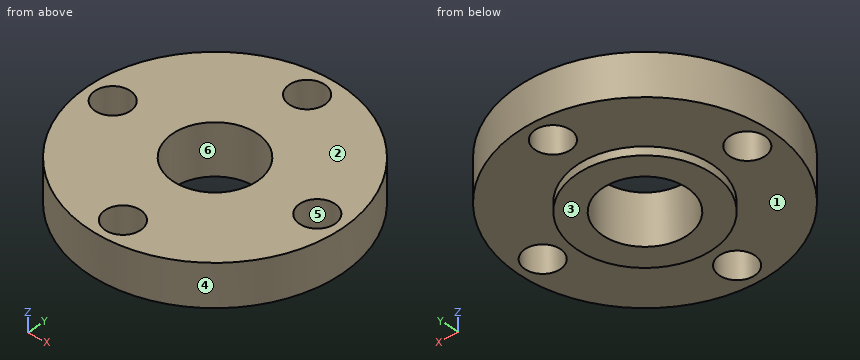
```python
from build123d import *

# Parameters (mm, degrees)
SKETCH1_R           = 15
BOSS_EXTRUDE1_DEPTH = 5
SKETCH2_R           = 2.1
CUT_EXTRUDE1_DEPTH  = 22.794494718
CIRPATTERN1_COUNT   = 4
SKETCH3_R           = 8
BOSS_EXTRUDE2_DEPTH = 1
SKETCH4_R           = 5
CUT_EXTRUDE3_DEPTH  = 23.045407685


with BuildPart() as part:
    # Sketch1 → Boss-Extrude1 (new body)
    with BuildSketch(Plane.XY):
        Circle(SKETCH1_R)
    extrude(amount=BOSS_EXTRUDE1_DEPTH)

    # Sketch2 → Cut-Extrude1 (cut, through all)
    with BuildSketch(Plane.XY.offset(5)):
        with Locations((0, 12)):
            Circle(SKETCH2_R)
    cut_extrude1 = extrude(amount=-CUT_EXTRUDE1_DEPTH, mode=Mode.SUBTRACT)

    # CirPattern1: Cut-Extrude1 ×4 about axis
    cirpattern1_axis = Axis((0, 0, 0), (0, 0, 1))
    for i in range(1, CIRPATTERN1_COUNT):
        add(cut_extrude1.rotate(cirpattern1_axis, i * 360 / CIRPATTERN1_COUNT), mode=Mode.SUBTRACT)

    # Sketch3 → Boss-Extrude2 (add)
    with BuildSketch(Plane(origin=(0, 0, 0), x_dir=(-1, 0, 0), z_dir=(0, 0, -1))):
        with Locations(Location((0, 0, 0), (0, 0, 180))):
            Circle(SKETCH3_R)
    extrude(amount=BOSS_EXTRUDE2_DEPTH)

    # Sketch4 → Cut-Extrude3 (cut, through all)
    with BuildSketch(Plane.XY.offset(5)):
        Circle(SKETCH4_R)
    extrude(amount=-CUT_EXTRUDE3_DEPTH, mode=Mode.SUBTRACT)


solid = part.part
```
For this review, take the finished solid that the model builds, in its own axes (mm). Face numbers are marked on the shaded views. A direction names the side the tool comes from. Give positions to 0.01 mm unless a question says otherwise; leave off trailing zeros. Order: outer loops, then holes, each group sorted by start corner. A loop starts at its lowest first (then second) coordinate and runs counter-clockwise, first axis right, second up.
1) The part is to be moulded in two halves that separate along X. For the marked faces 3, 4, 5 and 6, say which applies: released by +X, released by -X, zero draft, split by the parting line, or undercut.
2) Insertion check: pin 1 (2.5 mm diameter, centred on x = 0, y = 12, fed in from -Z); pin 2 (3 mm diameter, centred on y = 10, z = 0.5, fed in from -X); pin 3 (1.5 mm diameter, centred on y = -3.5, z = 3.5, fed in from +X); pin 4 (1.5 mm diameter, centred on y = 8.5, z = 1.5, fed in from -X). Each pin has a flat end and moves straight along its axis. Give the tip position at first contact, or say it passes through.
3) Take a section at B-B (y = 0). Give the boundary of the cut face in (x, z).
4) For the marked faces 1 and 2, list the 3-axis set-ups (+Z, -Z, +X, -X, +Y, -Y) from which the entire face can be reached by the end or side of a thin tool; tool diameter is ignored.
5) Take a section at C-C (x = 1). Give the boundary of the cut face in (y, z), then the cut area to 3 significant figures.
6) Take a section at A-A (x = -12). Give the boundary of the cut face in (y, z).
7) Wall thickness on line 1 (Y direction, x = 0, z = 3.1); line 2 (Y direction, x = 1.75, z = 0.85); line 3 (Y direction, x = 12.5, z = 2.2): over which ranges is each line inside the solid? List them lowest first.
Derived:
1. face 3: zero draft
1. face 4: split by the parting line
1. face 5: undercut
1. face 6: undercut
2. pin 1: passes through
2. pin 2: stops at x = -12.36
2. pin 3: stops at x = 14.75
2. pin 4: stops at x = -12.84
3. outline: (-15, 0) - (-14.1, 0) - (-14.1, 5) - (-15, 5) - close; (-9.9, 0) - (-8, 0) - (-8, -1) - (-5, -1) - (-5, 5) - (-9.9, 5) - close; (5, -1) - (8, -1) - (8, 0) - (9.9, 0) - (9.9, 5) - (5, 5) - close; (14.1, 0) - (15, 0) - (15, 5) - (14.1, 5) - close
4. face 1: -Z
4. face 2: +Z, +X, -X, +Y, -Y
5. outline: (-14.97, 0) - (-13.85, 0) - (-13.85, 5) - (-14.97, 5) - close; (-10.15, 0) - (-7.94, 0) - (-7.94, -1) - (-4.9, -1) - (-4.9, 5) - (-10.15, 5) - close; (4.9, -1) - (7.94, -1) - (7.94, 0) - (10.15, 0) - (10.15, 5) - (4.9, 5) - close; (13.85, 0) - (14.97, 0) - (14.97, 5) - (13.85, 5) - close
5. area: 69.8 mm2
6. outline: (-9, 0) - (-2.1, 0) - (-2.1, 5) - (-9, 5) - close; (2.1, 0) - (9, 0) - (9, 5) - (2.1, 5) - close
7. line 1: y = -15 to -14.1, -9.9 to -5, 5 to 9.9, 14.1 to 15
7. line 2: y = -14.9 to -13.16, -10.84 to -4.68, 4.68 to 10.84, 13.16 to 14.9
7. line 3: y = -8.29 to -2.04, 2.04 to 8.29
